```python
from build123d import *

# Parameters (mm, degrees)
SKETCH_1_R          = 25
EXTRUDE_1_DEPTH     = 27
SKETCH_2_R          = 16
CUT_EXTRUDE_1_DEPTH = 17
SKETCH_3_R          = 14
CUT_EXTRUDE_2_DEPTH = 40.230090492
CHAMFER_1_SIZE      = 1
CHAMFER_2_SIZE      = 0.5
SKETCH_4_W          = 2
SKETCH_4_H          = 1.3


with BuildPart() as part:
    # 草图1 → 凸台-拉伸1 (new body)
    with BuildSketch(Plane(origin=(0, 0, 0), x_dir=(1, 0, 0), z_dir=(0, 1, 0))):
        with Locations(Location((0, 0, 0), (0, 0, 270))):
            Circle(SKETCH_1_R)
    extrude(amount=EXTRUDE_1_DEPTH)

    # 草图2 → 切除-拉伸1 (cut)
    with BuildSketch(Plane(origin=(0, 27, 0), x_dir=(1, 0, 0), z_dir=(0, 1, 0))):
        with Locations(Location((0, 0, 0), (0, 0, 270))):
            Circle(SKETCH_2_R)
    extrude(amount=-CUT_EXTRUDE_1_DEPTH, mode=Mode.SUBTRACT)

    # 草图3 → 切除-拉伸2 (cut, through all)
    with BuildSketch(Plane(origin=(0, 10, 0), x_dir=(1, 0, 0), z_dir=(0, 1, 0))):
        with Locations(Location((0, 0, 0), (0, 0, 270))):
            Circle(SKETCH_3_R)
    extrude(amount=-CUT_EXTRUDE_2_DEPTH, mode=Mode.SUBTRACT)

    # 倒角1
    chamfer_1_edges = [part.edges().sort_by_distance(p)[0] for p in [
        (0, 0, -25),
        (0, 27, -25),
    ]]
    chamfer(chamfer_1_edges, length=CHAMFER_1_SIZE)

    # 倒角2
    chamfer_2_edges = [part.edges().sort_by_distance(p)[0] for p in [
        (0, 27, -16),
    ]]
    chamfer(chamfer_2_edges, length=CHAMFER_2_SIZE)

    # 草图4 → 切除-旋转1 (revolve, cut)
    with BuildSketch(Plane(origin=(0, 0, 0), x_dir=(0, 0, -1), z_dir=(1, 0, 0))):
        with Locations((-15.85, 17.65)):
            Rectangle(SKETCH_4_W, SKETCH_4_H)
    revolve(axis=Axis((0, 27, 0), (0, -1, 0)), mode=Mode.SUBTRACT)


solid = part.part
```
Part model, mm, in its own coordinate system. A direction names the side the tool comes from. Round coordinates to 2 decimals unless told otherwise and drop trailing zeros. Write each loop counter-clockwise with the first axis right and the second up, starting at its lowest first coordinate (ties: lowest second). Pieces come first, ordered by that corner, then holes. Notation, with made-up numbers: (65.5, -12.5) -> (71.5, -12.5) arc R30 ccw to (71.5, 22.5) -> close; hole circle Ø1 at (71.25, -14). An arc over 180 degrees is marked (long way). Return JSON: item names as keys, results as strings. Group by question number.
Q1. Saw through at B-B on y = 20.5. Write the cut outline in (x, z).
Q2. Saw through at C-C on y = 2.5. Write the cut outline in (x, z).
Q3. Saw through at A-A on z = 0. Write the cut outline in (x, y).
Q4. Probe L1, parallel to X at y = 23.75, z = 0; L2, parallel to X at y = 17.65, z = 0; L3, parallel to Z at x = -11, y = 22.5. List the from-to ranges inside material, lowest first. Write a range as [from, to].
Q5. Pin check, flat tips, straight feed: pin 1 (1 mm diameter, centred on y = 21.5, z = 14, fed in from +X); pin 2 (6 mm diameter, centred on y = 12.5, z = 12.5, fed in from +X); pin 3 (1 mm diameter, centred on x = 12.5, y = 7, fed in from -Z); pin 4 (17 mm diameter, centred on x = -3, z = 1, fed in from +Y). Stop position of each tip, or through.
Q6. Mould opens along Z. For faces 1 (the flat face through (-16, 27, -6)), 2 (the cylindrical face through (7.509, 13.325, 23.846)), 3 (the cylindrical face through (-16.707, 17.659, -2.194)) say: pulls with the +Z half, pulls with the -Z half, needs draft (parallel to the pull), parting line crosses it, or undercut.
Q7. Which spindle directions (+Z, -Z, +X, -X, +Y, -Y) get a long thin tool onto all of the face, cutting with end or side? Do faces 4 (the flat face through (6, 18.3, 15)), 5 (the cylindrical face through (-13.67, 5.07, -3.03)), 6 (the cylindrical face through (-15.62, 22.46, -3.47)). Say none if no direction does.
Answer:
{
 "1": {"outline": "circle Ø50 at (0, 0); hole circle Ø32 at (0, 0)"},
 "2": {"outline": "circle Ø50 at (0, 0); hole circle Ø28 at (0, 0)"},
 "3": {"outline": "(-25, 1) -> (-24, 0) -> (-14, 0) -> (-14, 10) -> (-16, 10) -> (-16, 17) -> (-16.85, 17) -> (-16.85, 18.3) -> (-16, 18.3) -> (-16, 26.5) -> (-16.5, 27) -> (-24, 27) -> (-25, 26) -> close; (14, 0) -> (24, 0) -> (25, 1) -> (25, 26) -> (24, 27) -> (16.5, 27) -> (16, 26.5) -> (16, 18.3) -> (16.85, 18.3) -> (16.85, 17) -> (16, 17) -> (16, 10) -> (14, 10) -> close"},
 "4": {"L1": "[-25, -16], [16, 25]", "L2": "[-25, -16.85], [16.85, 25]", "L3": "[-22.45, -11.62], [11.62, 22.45]"},
 "5": {"pin 1": "x = 21.04", "pin 2": "x = 23.12", "pin 3": "z = -21.93", "pin 4": "through"},
 "6": {"face 1": "needs draft", "face 2": "parting line crosses it", "face 3": "undercut"},
 "7": {"face 4": "none", "face 5": "+Y, -Y", "face 6": "+Y"}
}
